Verification items for the finished model (mm, model axes). Round coordinates to 2 decimals unless told otherwise and drop trailing zeros. Write each loop counter-clockwise with the first axis right and the second up, starting at its lowest first coordinate (ties: lowest second). Pieces come first, ordered by that corner, then holes. Notation, with made-up numbers: (18, 70.25) - (46, 70.25) arc R27 cw to (46, 105.25) - close; hole circle Ø11 at (45, 11.25). An arc over 180 degrees is marked (long way). Write each question's results on one line, items separated by ' | '.
```python
from build123d import *

# Parameters (mm, degrees)
SKETCH_1_W          = 8
SKETCH_1_H          = 8
SKETCH_1_W_2        = 6
SKETCH_1_H_2        = 6
EXTRUDE_1_DEPTH     = 185
SKETCH_2_R          = 1.55
CUT_EXTRUDE_1_DEPTH = 186.216090014
SKETCH_3_R          = 1.55
CUT_EXTRUDE_2_DEPTH = 186.216090014


with BuildPart() as part:
    # 草图1 → 凸台-拉伸1 (new body)
    with BuildSketch(Plane.XY):
        Rectangle(SKETCH_1_W, SKETCH_1_H)
        Rectangle(SKETCH_1_W_2, SKETCH_1_H_2, mode=Mode.SUBTRACT)
    extrude(amount=EXTRUDE_1_DEPTH)

    # 草图2 → 切除-拉伸1 (cut, through all)
    with BuildSketch(Plane(origin=(4, 0, 0), x_dir=(0, 0, -1), z_dir=(1, 0, 0))):
        with Locations(Location((-44.5, 0, 0), (0, 0, 90))):
            Circle(SKETCH_2_R)
        with Locations(Location((-60.5, 0, 0), (0, 0, 90))):
            Circle(SKETCH_2_R)
        with Locations(Location((-124.5, 0, 0), (0, 0, 90))):
            Circle(SKETCH_2_R)
        with Locations(Location((-140.5, 0, 0), (0, 0, 90))):
            Circle(SKETCH_2_R)
    extrude(amount=-CUT_EXTRUDE_1_DEPTH, mode=Mode.SUBTRACT)

    # 草图3 → 切除-拉伸2 (cut, through all)
    with BuildSketch(Plane(origin=(0, 4, 0), x_dir=(1, 0, 0), z_dir=(0, 1, 0))):
        with Locations(Location((0, -4, 0), (0, 0, 270))):
            Circle(SKETCH_3_R)
        with Locations(Location((0, -12, 0), (0, 0, 270))):
            Circle(SKETCH_3_R)
        with Locations(Location((0, -173, 0), (0, 0, 270))):
            Circle(SKETCH_3_R)
        with Locations(Location((0, -181, 0), (0, 0, 270))):
            Circle(SKETCH_3_R)
        with Locations(Location((0, -87.5, 0), (0, 0, 270))):
            Circle(SKETCH_3_R)
        with Locations(Location((0, -97.5, 0), (0, 0, 270))):
            Circle(SKETCH_3_R)
        with Locations(Location((0, -148, 0), (0, 0, 270))):
            Circle(SKETCH_3_R)
        with Locations(Location((0, -37, 0), (0, 0, 270))):
            Circle(SKETCH_3_R)
    extrude(amount=-CUT_EXTRUDE_2_DEPTH, mode=Mode.SUBTRACT)


solid = part.part
```
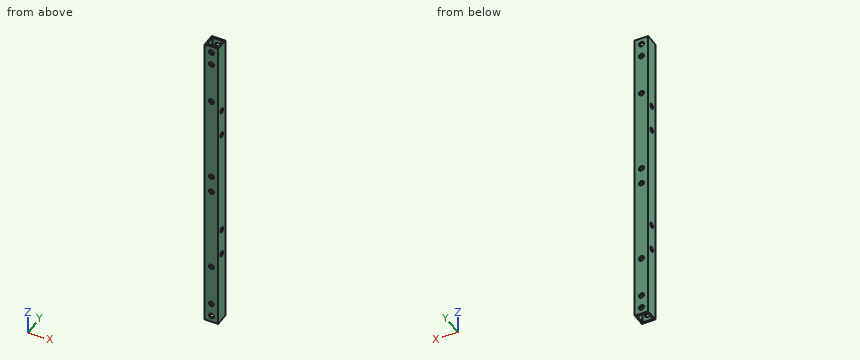
(1) Section check C-C (x = 0). State how many separate pieces and enclosed holes the cut face has, plus the area to 3 significant figures.
Answer:
separate pieces: 18 | enclosed holes: 0 | area: 320 mm2
(2) Section check A-A (z = 173). Record the cut outline in (x, y), plus the area to 3 significant figures.
Answer:
outline: (-4, -4) - (-1.55, -4) - (-1.55, -3) - (-3, -3) - (-3, 3) - (-1.55, 3) - (-1.55, 4) - (-4, 4) - close; (1.55, -4) - (4, -4) - (4, 4) - (1.55, 4) - (1.55, 3) - (3, 3) - (3, -3) - (1.55, -3) - close | area: 21.8 mm2
(3) Section check B-B (z = 54). Record the cut outline in (x, y), plus the area to 3 significant figures.
Answer:
outline: (-4, -4) - (4, -4) - (4, 4) - (-4, 4) - close; hole (-3, -3) - (3, -3) - (3, 3) - (-3, 3) - close | area: 28.0 mm2
(4) Thickness scan on L1, parallel to Z at x = -3.65, y = 0; L2, parallel to Y at x = -2.5, z = 140.5; L3, parallel to X at y = 3.8, z = 4. Record the ranges inside material, lowest first.
Answer:
L1: 0 to 42.95, 46.05 to 58.95, 62.05 to 122.95, 126.05 to 138.95, 142.05 to 185 | L2: -4 to -3, 3 to 4 | L3: -4 to -1.55, 1.55 to 4
(5) Go/stop test with flat-tipped pins: pin 1 Ø1.9 at (x, z) = (0, 4) entering from +Y; pin 2 Ø3 at (x, y) = (-2.5, 0.5) entering from -Z. Record where each tip stops, or that it passes through.
Answer:
pin 1: through | pin 2: z = 0
